from build123d import *

# Parameters (mm, degrees)
BOSS_EXTRUDE1_DEPTH                                  = 50
CUT_EXTRUDE1_REACH                                   = 92.995
SKETCH2_R                                            = 2.75
CUT_EXTRUDE2_REACH                                   = 87.837
HOLE_SIZE_PER_SOCKET_HEAD_CAP_SCREW_TYPE_D           = 6.6
HOLE_SIZE_PER_SOCKET_HEAD_CAP_SCREW_TYPE_DEPTH       = 34
HOLE_SIZE_PER_SOCKET_HEAD_CAP_SCREW_TYPE_CBORE_D     = 11
HOLE_SIZE_PER_SOCKET_HEAD_CAP_SCREW_TYPE_CBORE_DEPTH = 6.8
M6_TAPPED_HOLE1_D                                    = 5
CHAMFER1_SIZE                                        = 1


with BuildPart() as part:
    # Sketch1 → Boss-Extrude1 (new body)
    with BuildSketch(Plane.XY):
        Polygon((32, 10), (44, 10), (44, 0), (0, 0), (0, 10), (12, 10), (12, 62), (32, 62), align=None)
    extrude(amount=BOSS_EXTRUDE1_DEPTH)

    # Sketch2 → Cut-Extrude1 (cut, up to next)
    with BuildSketch(Plane.XZ, mode=Mode.PRIVATE) as cut_extrude1_sk1:
        with Locations(Location((6, 43, 0), (0, 0, 270))):
            Circle(SKETCH2_R)
    cut_extrude1_tool1 = extrude(cut_extrude1_sk1.sketch, amount=-CUT_EXTRUDE1_REACH, mode=Mode.PRIVATE) & part.part
    # Sketch2 → Cut-Extrude1 (cut, up to next)
    with BuildSketch(Plane.XZ, mode=Mode.PRIVATE) as cut_extrude1_sk2:
        with Locations(Location((6, 7, 0), (0, 0, 270))):
            Circle(SKETCH2_R)
    cut_extrude1_tool2 = extrude(cut_extrude1_sk2.sketch, amount=-CUT_EXTRUDE1_REACH, mode=Mode.PRIVATE) & part.part
    # Sketch2 → Cut-Extrude1 (cut, up to next)
    with BuildSketch(Plane.XZ, mode=Mode.PRIVATE) as cut_extrude1_sk3:
        with Locations(Location((38, 43, 0), (0, 0, 270))):
            Circle(SKETCH2_R)
    cut_extrude1_tool3 = extrude(cut_extrude1_sk3.sketch, amount=-CUT_EXTRUDE1_REACH, mode=Mode.PRIVATE) & part.part
    # Sketch2 → Cut-Extrude1 (cut, up to next)
    with BuildSketch(Plane.XZ, mode=Mode.PRIVATE) as cut_extrude1_sk4:
        with Locations(Location((38, 7, 0), (0, 0, 270))):
            Circle(SKETCH2_R)
    cut_extrude1_tool4 = extrude(cut_extrude1_sk4.sketch, amount=-CUT_EXTRUDE1_REACH, mode=Mode.PRIVATE) & part.part
    add(cut_extrude1_tool1.solids().sort_by_distance((6, 0, 43))[0], mode=Mode.SUBTRACT)
    add(cut_extrude1_tool2.solids().sort_by_distance((6, 0, 7))[0], mode=Mode.SUBTRACT)
    add(cut_extrude1_tool3.solids().sort_by_distance((38, 0, 43))[0], mode=Mode.SUBTRACT)
    add(cut_extrude1_tool4.solids().sort_by_distance((38, 0, 7))[0], mode=Mode.SUBTRACT)

    # Sketch3 → Cut-Extrude2 (cut, up to next)
    with BuildSketch(Plane.ZY.offset(-12), mode=Mode.PRIVATE) as cut_extrude2_sk1:
        with BuildLine():
            Line((34, 49.949874371), (34, 62))
            Line((34, 62), (36, 62))
            Line((36, 62), (36, 49.949874371))
            ThreePointArc((36, 49.949874371), (45, 40), (36, 30.050125629))
            Line((36, 30.050125629), (36, 27))
            Line((36, 27), (34, 27))
            Line((34, 27), (34, 30.050125629))
            ThreePointArc((34, 30.050125629), (25, 40), (34, 49.949874371))
        make_face()
    cut_extrude2_tool1 = extrude(cut_extrude2_sk1.sketch, amount=-CUT_EXTRUDE2_REACH, mode=Mode.PRIVATE) & part.part
    # Sketch3 → Cut-Extrude2 (cut, up to next)
    with BuildSketch(Plane.ZY.offset(-12), mode=Mode.PRIVATE) as cut_extrude2_sk2:
        Polygon((5, 26), (5, 29), (10, 29), (10, 11), (5, 11), (5, 14), (0, 14), (0, 26), align=None)
    cut_extrude2_tool2 = extrude(cut_extrude2_sk2.sketch, amount=-CUT_EXTRUDE2_REACH, mode=Mode.PRIVATE) & part.part
    add(cut_extrude2_tool1.solids().sort_by_distance((12, 40.915096, 35))[0], mode=Mode.SUBTRACT)
    add(cut_extrude2_tool2.solids().sort_by_distance((12, 20, 5.5))[0], mode=Mode.SUBTRACT)

    # Hole size per socket head cap screw type 1
    with Locations(Plane(origin=(0, 0, 0), x_dir=(-1, 0, 0), z_dir=(0, 0, -1))):
        with Locations((-22, 55)):
            CounterBoreHole(HOLE_SIZE_PER_SOCKET_HEAD_CAP_SCREW_TYPE_D / 2, HOLE_SIZE_PER_SOCKET_HEAD_CAP_SCREW_TYPE_CBORE_D / 2, HOLE_SIZE_PER_SOCKET_HEAD_CAP_SCREW_TYPE_CBORE_DEPTH, depth=HOLE_SIZE_PER_SOCKET_HEAD_CAP_SCREW_TYPE_DEPTH)

    # M6 Tapped Hole1 (through all)
    with Locations(Plane(origin=(0, 0, 0), x_dir=(-1, 0, 0), z_dir=(0, 0, -1))):
        with Locations((-22, 55)):
            Hole(M6_TAPPED_HOLE1_D / 2)

    # Chamfer1
    chamfer1_edges = [part.edges().sort_by_distance(p)[0] for p in [
        (44, 5, 50),
        (0, 5, 0),
        (22, 62, 50),
        (0, 5, 50),
        (22, 62, 0),
        (44, 5, 0),
    ]]
    chamfer(chamfer1_edges, length=CHAMFER1_SIZE)


solid = part.part
The listing builds one solid part. Answer for the finished solid, in the listing's coordinates (mm). A direction names the side the tool comes from. Coordinates: 2 decimals unless noted, no trailing zeros. Loops run counter-clockwise (first coordinate to the right, second up) from the corner with the lowest first, then second, coordinate; pieces in that order, holes last. Notation, with made-up numbers: (9, 9.25) -> (60, 9.25) arc R27 cw to (60, 47.25) -> close; hole circle Ø10 at (-14, -6). An arc over 180 degrees is marked (long way). Answer in a Markdown table with one row per item. Add a question column.
1. Flat-ended cylindrical pins translate along their axes: P1, Ø6, axis at x = 7, z = 36.5, coming from the +Y side; P2, Ø0.6, axis at x = 24, z = 34.5, coming from the +Y side; P3, Ø3, axis at y = 42, z = 5.5, coming from the +X side. Find the tip coordinate at first contact, or state that the pin passes through.
2. The part is cut by section C-C, the plane z = 37. Write down the section's boundary in (x, y).
3. The part is cut by section A-A, the plane z = 43. Write down the section's boundary in (x, y).
4. The part is cut by section B-B, the plane x = 22. Count the separate pieces of the cut face and the enclosed holes in it, then the cut area to 3 significant figures.
5. The part is cut by section D-D, the plane y = 47.5. Write down the section's boundary in (x, z).
6. For faces 5 (the flat face through (22, 29, 36)), 6 (the flat face through (22, 14, 3)), 7 (the cylindrical face through (22, 40, 25)), determine the directions among +Z, -Z, +X, -X, +Y, -Y from which every point of the face is accessible in a straight line to the end or side of a thin tool.
7. Determine the mould class of faces 1 (the cylindrical face through (4.95, 4.93, 4.46)), 2 (the flat face through (0, 5, 25)), 3 (the cylindrical face through (23.774, 57.783, 20.59)), 4 (the flat face through (38, 10, 25)) for opening direction X: +X half, -X half, draft (parallel to the pull), parting line (faces both ways), or undercut.
8. Consider line 1 (X direction, y = 7.75, z = 7); line 2 (Z direction, x = 17.5, y = 55); line 3 (Y direction, x = 12.5, z = 4). Determine where each line is inside the solid, lowest interval first. Write a range as [from, to].
Answer below:
| question | item | result |
|---|---|---|
| 1 | P1 | y = 10 |
| 1 | P2 | y = 27 |
| 1 | P3 | x = 32 |
| 2 | outline | (0, 0) -> (44, 0) -> (44, 10) -> (32, 10) -> (32, 30.2) -> (12, 30.2) -> (12, 10) -> (0, 10) -> close; (12, 49.8) -> (32, 49.8) -> (32, 62) -> (12, 62) -> close; hole circle Ø5 at (22, 55) |
| 3 | outline | (0, 0) -> (3.25, 0) -> (3.25, 10) -> (0, 10) -> close; (8.75, 0) -> (35.25, 0) -> (35.25, 10) -> (32, 10) -> (32, 34) -> (12, 34) -> (12, 10) -> (8.75, 10) -> close; (12, 46) -> (32, 46) -> (32, 62) -> (12, 62) -> close; (40.75, 0) -> (44, 0) -> (44, 10) -> (40.75, 10) -> close; hole circle Ø5 at (22, 55) |
| 4 | separate pieces | 3 |
| 4 | enclosed holes | 0 |
| 4 | area | 2,280 mm2 |
| 5 | outline | (12, 0) -> (32, 0) -> (32, 28.39) -> (12, 28.39) -> close; (12, 41.61) -> (32, 41.61) -> (32, 50) -> (12, 50) -> close |
| 6 | face 5 | +X, -X, +Y |
| 6 | face 6 | -Z, +X, -X |
| 6 | face 7 | +X, -X |
| 7 | face 1 | undercut |
| 7 | face 2 | -X half |
| 7 | face 3 | undercut |
| 7 | face 4 | draft |
| 8 | line 1 | [0, 3.25], [8.75, 35.25], [40.75, 44] |
| 8 | line 2 | [6.8, 34], [36, 50] |
| 8 | line 3 | [0, 14], [26, 62] |
